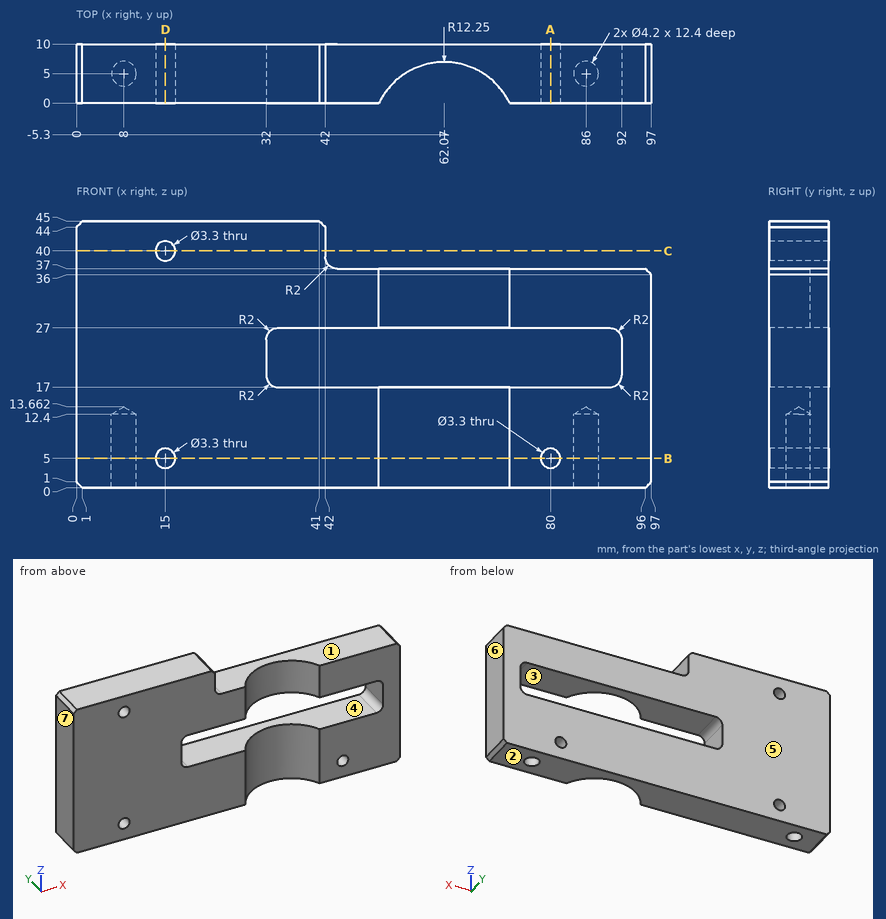
Study the drawing (mm; zero at the part's minimum x, y, z) and answer. A direction names the side the tool comes from. Coordinates: 2 decimals unless noted, no trailing zeros. Write each loop counter-clockwise with the first axis right and the second up, starting at its lowest first coordinate (ties: lowest second). Pieces come first, ordered by that corner, then holes.
Q1. Determine the mould class of the marked faces 4, 5, 6 and 7 for opening direction X: released by +X, released by -X, zero draft, split by the parting line, or undercut.
Q2. Which of the six approach directions +Z, -Z, +X, -X, +Y, -Y give full straight-line access (tool end or side, diameter ignored) to the marked faces 1, 2 and 3?
Q3. A cutting plane is placed at A-A, the plane x = 80. Give the vertices of the cut face in (y, z), then the cut area to 3 significant figures.
Q4. A cutting plane is placed at B-B, the plane z = 5. Give the vertices of the cut face in (x, y).
Q5. Each of these flat-tipped pins is pushed along its axis until it touches: pin 1 Ø3 at (x, z) = (80, 5) entering from +Y; pin 2 Ø4 at (y, z) = (4.5, 41.5) entering from +X; pin 3 Ø2.5 at (x, y) = (86, 5) entering from +Z. Where does it stop, or does it pass through?
Q6. A cutting plane is placed at C-C, the plane z = 40. Give the vertices of the cut face in (x, y).
Q7. A cutting plane is placed at D-D, the plane x = 15. Give the vertices of the cut face in (y, z), then the cut area to 3 significant figures.
Q8. Find the intervals of material crossed by line 1 (X direction, y = 6.75, z = 40); line 2 (Z direction, x = 38, y = 6.25); line 3 (Z direction, x = 87, y = 1), in increasing order.
Findings below:
1. face 4: undercut
1. face 5: zero draft
1. face 6: released by +X
1. face 7: released by -X
2. face 1: +Z, +X, +Y, -Y
2. face 2: -Z, +X, -X, +Y, -Y
2. face 3: +Y, -Y
3. outline: (0, 0) - (10, 0) - (10, 3.35) - (0, 3.35) - close; (0, 6.65) - (10, 6.65) - (10, 17) - (0, 17) - close; (0, 27) - (10, 27) - (10, 37) - (0, 37) - close
3. area: 237 mm2
4. outline: (0, 0) - (13.35, 0) - (13.35, 10) - (0, 10) - close; (16.65, 0) - (51.03, 0) arc R12.25 cw to (73.11, 0) - (78.35, 0) - (78.35, 10) - (16.65, 10) - close; (81.65, 0) - (97, 0) - (97, 10) - (81.65, 10) - close; hole circle Ø4.2 at (8, 5); hole circle Ø4.2 at (86, 5)
5. pin 1: passes through
5. pin 2: stops at x = 42
5. pin 3: stops at z = 37
6. outline: (0, 0) - (13.35, 0) - (13.35, 10) - (0, 10) - close; (16.65, 0) - (42, 0) - (42, 10) - (16.65, 10) - close
7. outline: (0, 0) - (10, 0) - (10, 3.35) - (0, 3.35) - close; (0, 6.65) - (10, 6.65) - (10, 38.35) - (0, 38.35) - close; (0, 41.65) - (10, 41.65) - (10, 45) - (0, 45) - close
7. area: 384 mm2
8. line 1: x = 0 to 13.35, 16.65 to 42
8. line 2: z = 0 to 17, 27 to 45
8. line 3: z = 0 to 17, 27 to 37
